```python
from build123d import *

# Parameters (mm, degrees)
FILLET1_R = 10


with BuildPart() as part:
    # Sketch1 → Revolve1 (revolve)
    with BuildSketch(Plane.XY, mode=Mode.PRIVATE) as revolve1_sk:
        Polygon((0, 0), (0, 370), (150, 370), (150, 70), (20, 70), (20, 30), (15, 30), (15, 0), align=None)
    revolve(revolve1_sk.sketch.rotate(Axis((0, 0, 0), (0, 1, 0)), 90), axis=Axis((0, 0, 0), (0, 1, 0)))

    # Fillet1
    fillet1_edges = [part.edges().sort_by_distance(p)[0] for p in [
        (0, 70, 150),
        (0, 370, 150),
    ]]
    fillet(fillet1_edges, radius=FILLET1_R)


solid = part.part
```
For this review, take the finished solid that the model builds, in its own axes (mm). A direction names the side the tool comes from. Round coordinates to 2 decimals unless told otherwise and drop trailing zeros. Write each loop counter-clockwise with the first axis right and the second up, starting at its lowest first coordinate (ties: lowest second). Pieces come first, ordered by that corner, then holes. Notation, with made-up numbers: (-13.5, 33.5) - (20.5, 33.5) arc R19 cw to (20.5, 62.5) - close; hole circle Ø10 at (18.25, 73). An arc over 180 degrees is marked (long way). Answer as a JSON object with one key per item and string values.
1. Draft analysis for pull direction Y (two halves, no side actions). For faces 1 (the face through (-2, 370, -2)), 2 (the face through (0, 0, 0)), 3 (the face through (-0.88, 49.72, 19.98)), state which applies: +Y half, -Y half, draft (parallel to the pull), parting line (faces both ways), or undercut.
Response values:
{"face 1": "+Y half", "face 2": "-Y half", "face 3": "draft"}
2. We need section D-D on y = 139.5. Give the boundary of the cut face in (x, z), then the cut area to 3 significant figures.
Response values:
{"outline": "circle Ø300 at (0, 0)", "area": "70,700 mm2"}
3. Tool access review of faces 4 (the face through (133.076, 218.04, -69.216)), 5 (the face through (-15, 30, -3)): name each direction out of +Z, -Z, +X, -X, +Y, -Y from which nothing blocks a thin tool from reaching the whole face with its end or side.
Response values:
{"face 4": "+Y, -Y", "face 5": "-Y"}
4. To check wall thickness, follow line 1 along Y through (x, z) = (-76, -19); line 2 along X through (y, z) = (277, -3); line 3 along X through (y, z) = (169, 64). State the ranges of each line that lie inside material, in increasing order.
Response values:
{"line 1": "y = 70 to 370", "line 2": "x = -149.97 to 149.97", "line 3": "x = -135.66 to 135.66"}
5. We need section A-A on z = 0. Give the boundary of the cut face in (x, y).
Response values:
{"outline": "(-150, 80) arc R10 ccw to (-140, 70) - (-20, 70) - (-20, 30) - (-15, 30) - (-15, 0) - (15, 0) - (15, 30) - (20, 30) - (20, 70) - (140, 70) arc R10 ccw to (150, 80) - (150, 360) arc R10 ccw to (140, 370) - (-140, 370) arc R10 ccw to (-150, 360) - close"}
6. We need section C-C on y = 23.5. Give the boundary of the cut face in (x, z).
Response values:
{"outline": "circle Ø30 at (0, 0)"}
7. For pin 1 Ø12 at (y, z) = (318, -16.5) entering from -X; pin 2 Ø12 at (x, z) = (-82.5, -16.5) entering from -Y; pin 3 Ø10 at (x, y) = (-18, 173.5) entering from -Z, all flat-tipped, find the tip position at first contact; note any pin that passes through.
Response values:
{"pin 1": "stops at x = -149.63", "pin 2": "stops at y = 70", "pin 3": "stops at z = -149.44"}
8. We need section B-B on x = 0. Give the boundary of the cut face in (y, z), then the cut area to 3 significant figures.
Response values:
{"outline": "(0, -15) - (30, -15) - (30, -20) - (70, -20) - (70, -140) arc R10 ccw to (80, -150) - (360, -150) arc R10 ccw to (370, -140) - (370, 140) arc R10 ccw to (360, 150) - (80, 150) arc R10 ccw to (70, 140) - (70, 20) - (30, 20) - (30, 15) - (0, 15) - close", "area": "92,400 mm2"}
